Check sheet for the modelled part. Datum: model origin and axes. Units: mm. Coordinates: 2 decimals unless noted, no trailing zeros. Write each loop counter-clockwise with the first axis right and the second up, starting at its lowest first coordinate (ties: lowest second). Pieces come first, ordered by that corner, then holes. Notation, with made-up numbers: (-30.75, 62) -> (-4.75, 62) arc R34 cw to (-4.75, 99) -> close; hole circle Ø6 at (63, 46.5). An arc over 180 degrees is marked (long way). Put each result on its own line as item: value.
```python
from build123d import *

# Parameters (mm, degrees)
BOSS_EXTRUDE1_DEPTH = 7.5


with BuildPart() as part:
    # Sketch1 → Boss-Extrude1 (new, symmetric)
    with BuildSketch(Plane.XY):
        Polygon((0, 0), (0, 10), (40, 50), (50, 50), (50, 10), (40, 0), align=None)
    extrude(amount=BOSS_EXTRUDE1_DEPTH, both=True)


solid = part.part
```
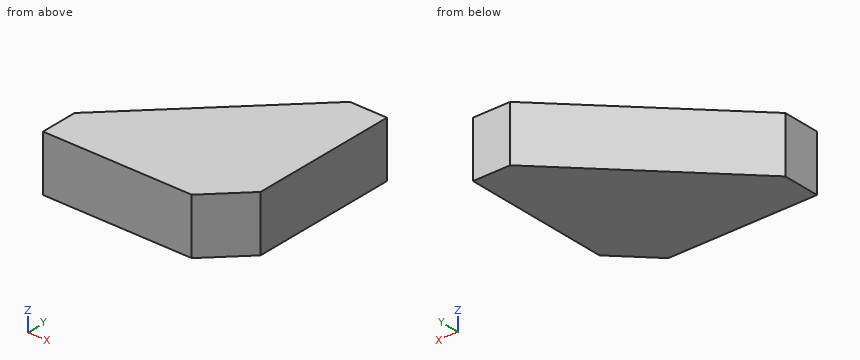
Q1. Cross-section at B-B (x = 7.5). Record the cut outline in (y, z).
Recorded:
outline: (0, -7.5) -> (17.5, -7.5) -> (17.5, 7.5) -> (0, 7.5) -> close
Q2. Material ranges on line 1 along X through (y, z) = (20, 5.25); line 2 along Y through (x, z) = (29.5, 0.75); line 3 along Y through (x, z) = (28, 0.25), recorded low to high.
Recorded:
line 1: x = 10 to 50
line 2: y = 0 to 39.5
line 3: y = 0 to 38
Q3. Cross-section at C-C (y = 28.5). Record the cut outline in (x, z), plus the area to 4 significant figures.
Recorded:
outline: (18.5, -7.5) -> (50, -7.5) -> (50, 7.5) -> (18.5, 7.5) -> close
area: 472.5 mm2
Q4. Cross-section at A-A (z = 0.5). Record the cut outline in (x, y).
Recorded:
outline: (0, 0) -> (40, 0) -> (50, 10) -> (50, 50) -> (40, 50) -> (0, 10) -> close
